Could you check a few things on this model? Use its own coordinates, in mm. Face numbers are marked on the shaded views. A direction names the side the tool comes from. Give positions to 0.01 mm unless a question says otherwise; leave off trailing zeros. Write each loop counter-clockwise with the first axis right and the second up, starting at its lowest first coordinate (ties: lowest second). Pieces come first, ordered by that corner, then holes. Notation, with made-up numbers: (7.5, 41) - (40.5, 41) arc R28 cw to (40.5, 62) - close; hole circle Ø6 at (13.5, -4.75). An arc over 180 degrees is marked (long way). Answer in a Markdown table with one row per item.
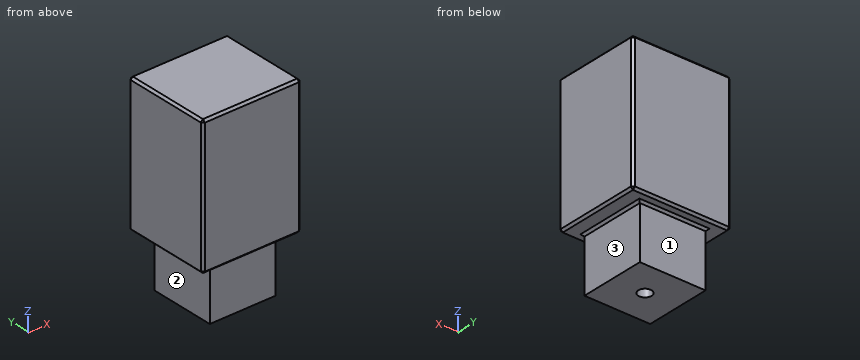
from build123d import *

# Parameters (mm, degrees)
SKETCH_1_W          = 60
SKETCH_1_H          = 60
EXTRUDE_227_DEPTH   = 50
SKETCH_2_W          = 90
SKETCH_2_H          = 80
EXTRUDE_1_DEPTH     = 125
CHAMFER_1_SIZE      = 2
SKETCH_3_R          = 6
CUT_EXTRUDE_1_DEPTH = 80


with BuildPart() as part:
    # 草图1 → Extrude 227 (new body)
    with BuildSketch(Plane.XY):
        with Locations((30, 30)):
            Rectangle(SKETCH_1_W, SKETCH_1_H)
    extrude(amount=EXTRUDE_227_DEPTH)

    # 草图2 → 凸台-拉伸1 (add)
    with BuildSketch(Plane.XY.offset(50)):
        with Locations((30, 30)):
            Rectangle(SKETCH_2_W, SKETCH_2_H)
    extrude(amount=EXTRUDE_1_DEPTH)

    # 倒角1
    chamfer_1_edges = [part.edges().sort_by_distance(p)[0] for p in [
        (-15, 70, 112.5),
        (75, 70, 112.5),
        (30, 70, 50),
        (30, 70, 175),
        (-15, -10, 112.5),
        (-15, 30, 50),
        (-15, 30, 175),
        (75, -10, 112.5),
        (75, 30, 50),
        (75, 30, 175),
        (30, -10, 50),
        (0, 30, 50),
        (30, 60, 50),
        (60, 30, 50),
        (30, 0, 50),
        (30, -10, 175),
    ]]
    chamfer(chamfer_1_edges, length=CHAMFER_1_SIZE)

    # 草图3 → 切除-拉伸1 (cut)
    with BuildSketch(Plane(origin=(0, 0, 0), x_dir=(-1, 0, 0), z_dir=(0, 0, -1))):
        with Locations((-30, 30)):
            Circle(SKETCH_3_R)
    extrude(amount=-CUT_EXTRUDE_1_DEPTH, mode=Mode.SUBTRACT)


solid = part.part
1) Imagine slicing it at D-D (y = 30). List the corners of the cut face in (x, z) for me, then the cut area to 3 significant figures.
Check values:
| item | result |
|---|---|
| outline | (-15, 52) - (-13, 50) - (-2, 50) - (0, 48) - (0, 0) - (24, 0) - (24, 80) - (36, 80) - (36, 0) - (60, 0) - (60, 48) - (62, 50) - (73, 50) - (75, 52) - (75, 173) - (73, 175) - (-13, 175) - (-15, 173) - close |
| area | 13,300 mm2 |
2) Imagine slicing it at C-C (x = 30). List the corners of the cut face in (y, z) for me, then the cut area to 3 significant figures.
Check values:
| item | result |
|---|---|
| outline | (-10, 52) - (-8, 50) - (-2, 50) - (0, 48) - (0, 0) - (24, 0) - (24, 80) - (36, 80) - (36, 0) - (60, 0) - (60, 48) - (62, 50) - (68, 50) - (70, 52) - (70, 173) - (68, 175) - (-8, 175) - (-10, 173) - close |
| area | 12,000 mm2 |
3) If I drill on line 1 (Y direction, x = 30, z = 59); line 2 (Y direction, x = 30, z = 39); line 3 (X direction, y = 45, z = 34), over which ranges is the centre line in solid material (lowest first)?
Check values:
| item | result |
|---|---|
| line 1 | y = -10 to 24, 36 to 70 |
| line 2 | y = 0 to 24, 36 to 60 |
| line 3 | x = 0 to 60 |
4) Imagine slicing it at A-A (z = 69). List the corners of the cut face in (x, y) for me.
Check values:
| item | result |
|---|---|
| outline | (-15, -8) - (-13, -10) - (73, -10) - (75, -8) - (75, 68) - (73, 70) - (-13, 70) - (-15, 68) - close; hole circle Ø12 at (30, 30) |
5) Imagine slicing it at B-B (y = 41). List the corners of the cut face in (x, z) for me.
Check values:
| item | result |
|---|---|
| outline | (-15, 52) - (-13, 50) - (-2, 50) - (0, 48) - (0, 0) - (60, 0) - (60, 48) - (62, 50) - (73, 50) - (75, 52) - (75, 173) - (73, 175) - (-13, 175) - (-15, 173) - close |
6) Will these pins go through, and if not, where does the flat tip stop? P1, Ø5, axis at x = 15, z = 19.5, coming from the -Y side; P2, Ø1.5, axis at y = 56.5, z = 50, coming from the +X side; P3, Ø2, axis at x = 20, z = 45.5, coming from the +Y side.
Check values:
| item | result |
|---|---|
| P1 | stops at y = 0 |
| P2 | stops at x = 73.75 |
| P3 | stops at y = 60 |
7) On a 3-axis mill with a long thin cutter (end or side, diameter ignored), from which of +Z, -Z, +X, -X, +Y, -Y can I reach the whole of each face in a straight line? I mean the marked faces 1, 2 and 3. Say none if no direction works.
Check values:
| item | result |
|---|---|
| face 1 | -Z, +X, -X, +Y |
| face 2 | -Z, -X, +Y, -Y |
| face 3 | -Z, +X, +Y, -Y |
